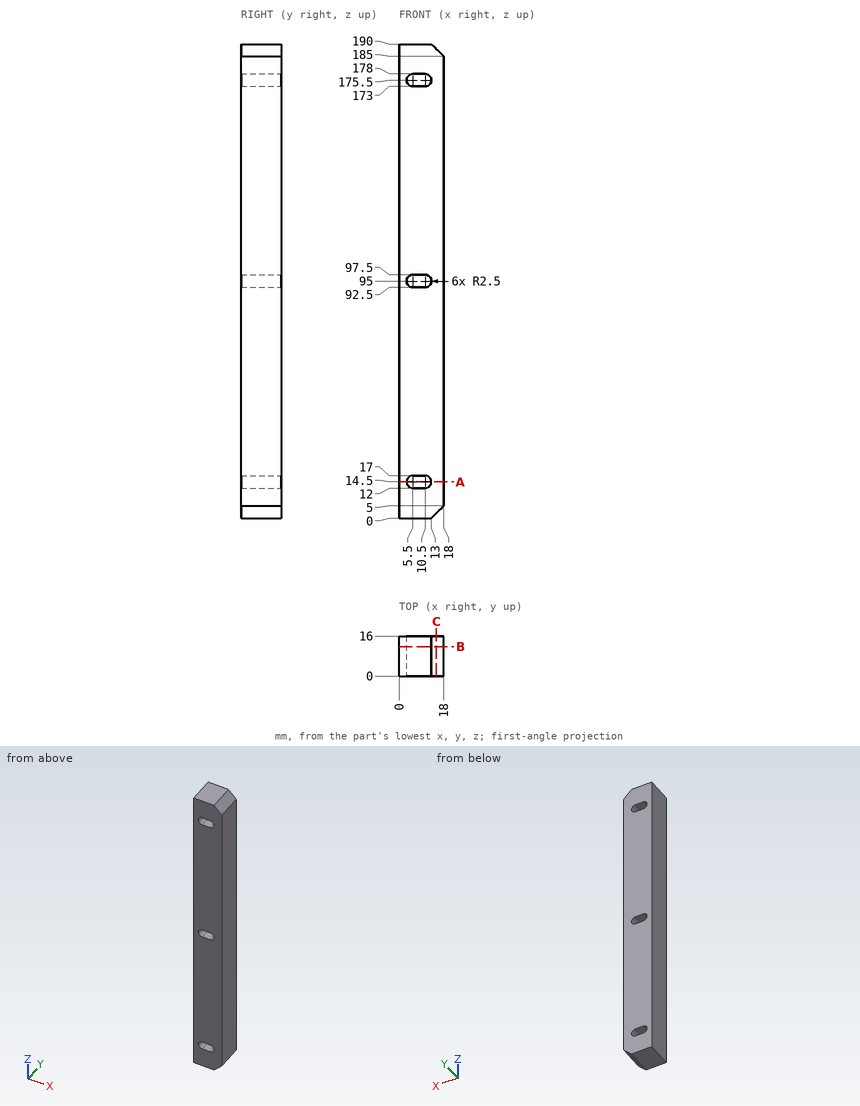
Input: dimensioned drawing with shaded views. Units: mm. Origin: part minimum x, y, z. Round coordinates to 2 decimals unless told otherwise and drop trailing zeros. Order: outer loops, then holes, each group sorted by start corner. A loop starts at its lowest first (then second) coordinate and runs counter-clockwise, first axis right, second up. Notation, with made-up numbers: (37.5, 48.25) -> (41.5, 48.25) arc R22 ccw to (41.5, 84.25) -> close; hole circle Ø4 at (65.25, 56). An arc over 180 degrees is marked (long way). One line per item, written item: value. Start each with the question number.
Q1. Section query A-A (z = 14.5). Return the cut outline in (x, y), plus the area to 3 significant figures.
Q2. Material intervals for probe 1 along Z at (x, y) = (8, 4.5); probe 2 along Z at (x, y) = (12.5, 2.25); probe 3 along X at (y, z) = (15.25, 176), sorted ascending.
Q3. Section query B-B (y = 11.75). Return the cut outline in (x, z).
Q4. Section query C-C (x = 15). Return the cut outline in (y, z).
Q5. Pin query (flat end, axial travel): pin 1 (1.5 mm diameter, centred on x = 14, y = 10, fed in from +Z). Return the tip coordinate at first contact, or that it passes through.
Findings below:
1. outline: (0, 0) -> (3, 0) -> (3, 16) -> (0, 16) -> close; (13, 0) -> (18, 0) -> (18, 16) -> (13, 16) -> close
1. area: 128 mm²
2. probe 1: 0 to 12, 17 to 92.5, 97.5 to 173, 178 to 190
2. probe 2: 0 to 13, 16 to 93.5, 96.5 to 174, 177 to 190
2. probe 3: 0 to 3.05, 12.95 to 18
3. outline: (0, 0) -> (13, 0) -> (18, 5) -> (18, 185) -> (13, 190) -> (0, 190) -> close; hole (5.5, 12) -> (10.5, 12) arc R2.5 ccw to (10.5, 17) -> (5.5, 17) arc R2.5 ccw to start; hole (5.5, 92.5) -> (10.5, 92.5) arc R2.5 ccw to (10.5, 97.5) -> (5.5, 97.5) arc R2.5 ccw to start; hole (5.5, 173) -> (10.5, 173) arc R2.5 ccw to (10.5, 178) -> (5.5, 178) arc R2.5 ccw to start
4. outline: (0, 2) -> (16, 2) -> (16, 188) -> (0, 188) -> close
5. pin 1: z = 189.75
